Source: CAD feature listing. Evaluate the final solid. Frame: model axes, mm. Face numbers are marked on the shaded views. A direction names the side the tool comes from. Round coordinates to 2 decimals unless told otherwise and drop trailing zeros. Order: outer loops, then holes, each group sorted by start corner. A loop starts at its lowest first (then second) coordinate and runs counter-clockwise, first axis right, second up. Notation, with made-up numbers: (72.25, 88.25) - (113.25, 88.25) arc R9 cw to (113.25, 101.25) - close; hole circle Ø3 at (89.5, 70). An arc over 180 degrees is marked (long way). Put each result on its own line as item: value. Start each with the question number.
1) Section A-A on y = 85.5. Output: boundary loops of the cut face in (x, z).
2) Section C-C on z = -48. Output: boundary loops of the cut face in (x, y), then the cut area to 3 significant figures.
3) Section B-B on x = 0. Output: boundary loops of the cut face in (y, z).
4) Access query for the marked faces 1, 2, 3 and 4. Directions: +Z, -Z, +X, -X, +Y, -Y. A direction counts if a zero-diameter tool reaches every point of the face in a straight line with its end or side. Return the directions, or none.
5) Section D-D on y = 17.5. Output: boundary loops of the cut face in (x, z), then the cut area to 3 significant figures.
6) Contact query for flat-ended pins moving along their axis: P1, Ø3, axis at x = -91.5, z = 1, coming from the +Y side; P2, Ø6, axis at y = 105, z = -61.5, coming from the -X side; P3, Ø15, axis at x = 12.5, y = 53.5, coming from the +Z side. Output: stop coordinate, or through.
7) Line query: probe 1 along Z at (x, y) = (21, 61); probe 2 along Y at (x, z) = (92, -11.5). Output: solid intervals per line, ascending. Write a range as [from, to].
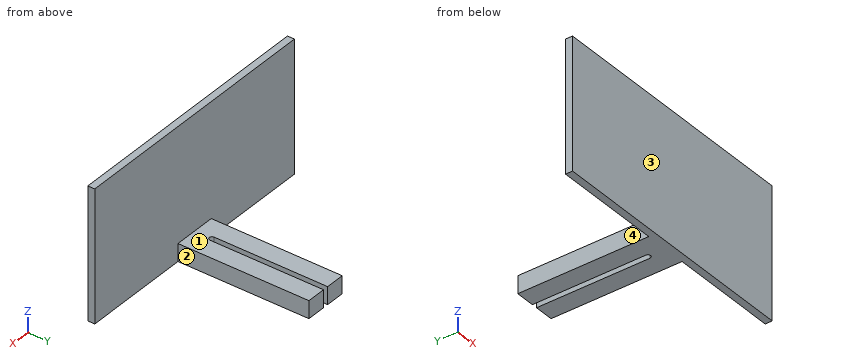
```python
from build123d import *

# Parameters (mm, degrees)
SKETCH1_W           = 300
SKETCH1_H           = 150
BOSS_EXTRUDE1_DEPTH = 8
SKETCH2_W           = 50
SKETCH2_H           = 20
BOSS_EXTRUDE2_DEPTH = 150
CUT_EXTRUDE1_DEPTH  = 254.700610957


with BuildPart() as part:
    # Sketch1 → Boss-Extrude1 (new body)
    with BuildSketch(Plane(origin=(0, 0, 0), x_dir=(1, 0, 0), z_dir=(0, 1, 0))):
        Rectangle(SKETCH1_W, SKETCH1_H)
    extrude(amount=BOSS_EXTRUDE1_DEPTH)

    # Sketch2 → Boss-Extrude2 (add)
    with BuildSketch(Plane(origin=(0, 8, 0), x_dir=(1, 0, 0), z_dir=(0, 1, 0))):
        with Locations((0, 65)):
            Rectangle(SKETCH2_W, SKETCH2_H)
    extrude(amount=BOSS_EXTRUDE2_DEPTH)

    # Sketch3 → Cut-Extrude1 (cut, through all)
    with BuildSketch(Plane.XY.offset(-55)):
        with BuildLine():
            Line((3.1, 158), (3.1, 28))
            ThreePointArc((3.1, 28), (0, 24.9), (-3.1, 28))
            Line((-3.1, 28), (-3.1, 158))
            ThreePointArc((-3.1, 158), (0, 161.1), (3.1, 158))
        make_face()
    extrude(amount=-CUT_EXTRUDE1_DEPTH, mode=Mode.SUBTRACT)


solid = part.part
```
Answer sheet:
1. outline: (-25, -75) - (-3.1, -75) - (-3.1, -55) - (-25, -55) - close; (3.1, -75) - (25, -75) - (25, -55) - (3.1, -55) - close
2. outline: (-150, 0) - (150, 0) - (150, 8) - (-150, 8) - close
2. area: 2,400 mm^2
3. outline: (0, -75) - (24.9, -75) - (24.9, -55) - (8, -55) - (8, 75) - (0, 75) - close
4. face 1: +Z, +X, -X, +Y
4. face 2: +Z, -Z, +X, +Y
4. face 3: +Z, -Z, +X, -X, -Y
4. face 4: +Z, -Z, -X, +Y
5. outline: (-25, -75) - (25, -75) - (25, -55) - (-25, -55) - close
5. area: 1,000 mm^2
6. P1: y = 8
6. P2: x = -25
6. P3: z = -55
7. probe 1: [-75, -55]
7. probe 2: [0, 8]
